```python
from build123d import *

# Parameters (mm, degrees)
BOSS_EXTRUDE1_DEPTH       = 9
BOSS_EXTRUDE1_DEPTH_BACK  = 9
SKETCH1_R                 = 5.25
M4X0_7_TAPPED_HOLE2_D     = 3.3
M4X0_7_TAPPED_HOLE2_DEPTH = 7.1
M4X0_7_TAPPED_HOLE2_TIP   = 0.991420021


with BuildPart() as part:
    # Sketch1 → Boss-Extrude1 (new, two sides: drawn at the far end of the back side and taken through both)
    with BuildSketch(Plane(origin=(0, 0, 0), x_dir=(1, 0, 0), z_dir=(0, 1, 0)).offset(-BOSS_EXTRUDE1_DEPTH_BACK)):
        with BuildLine():
            Line((0, 0), (0, -115))
            Line((0, -115), (2, -115))
            Line((2, -115), (14.5, -95))
            Line((14.5, -95), (30, 2.863148477))
            ThreePointArc((30, 2.863148477), (29.226286483, 10.190585207), (25.056843998, 16.265592284))
            Line((25.056843998, 16.265592284), (25.056843998, 40))
            ThreePointArc((25.056843998, 40), (16.056843998, 49), (7.056843998, 40))
            Line((7.056843998, 40), (7.056843998, 17.036728487))
            Line((7.056843998, 17.036728487), (0, 0))
        make_face()
        with Locations(Location((16.056843998, 40, 0), (0, 0, 270))):
            Circle(SKETCH1_R, mode=Mode.SUBTRACT)
        with Locations(Location((15.152984624, 5, 0), (0, 0, 270))):
            Circle(SKETCH1_R, mode=Mode.SUBTRACT)
    extrude(amount=BOSS_EXTRUDE1_DEPTH + BOSS_EXTRUDE1_DEPTH_BACK)

    # M4x0.7 Tapped Hole2
    with Locations(Plane(origin=(0, 0, 60), x_dir=(0, 0, -1), z_dir=(-1, 0, 0))):
        with Locations((0, 0), (-48, 0)):
            Hole(M4X0_7_TAPPED_HOLE2_D / 2, depth=M4X0_7_TAPPED_HOLE2_DEPTH)
            with Locations((0, 0, -(M4X0_7_TAPPED_HOLE2_DEPTH + M4X0_7_TAPPED_HOLE2_TIP / 2))):  # 118° drill point
                Cone(0, M4X0_7_TAPPED_HOLE2_D / 2, M4X0_7_TAPPED_HOLE2_TIP, mode=Mode.SUBTRACT)


solid = part.part
```
Work out the finished part from the listing and answer in its coordinate system (mm). A direction names the side the tool comes from. Give positions to 0.01 mm unless a question says otherwise; leave off trailing zeros. Order: outer loops, then holes, each group sorted by start corner. A loop starts at its lowest first (then second) coordinate and runs counter-clockwise, first axis right, second up. Notation, with made-up numbers: M 12.5,-32 L 25.5,-32 A14 cw 25.5,-14 Z; hole C -37.75,-1 d8. An arc over 180 degrees is marked long. Return JSON: item names as keys, results as strings.
1) Straight lines are drawn through the part: line 1 along Z through (x, y) = (4, 0.75); line 2 along Y through (x, z) = (3.75, 60); line 3 along Z through (x, y) = (13, -7.5). For each, find the intervals that lie inside material, in ascending order. Write a range as [from, to].
Resolved:
{"line 1": "[-9.66, 58.53], [61.47, 106.53], [109.47, 111.8]", "line 2": "[-9, -1.65], [1.65, 9]", "line 3": "[-48.46, -44.27], [-35.73, -9.79], [-0.21, 97.4]"}
2) Section A-A, the plane y = 6.5 is taken. Write down the section's boundary in (x, z), plus the area to 3 significant figures.
Resolved:
{"outline": "M 0,0 L 7.06,-17.04 L 7.06,-40 A9 ccw 25.06,-40 L 25.06,-16.27 A15 ccw 30,-2.86 L 14.5,95 L 2,115 L 0,115 Z; hole C 15.15,-5 d10.5; hole C 16.06,-40 d10.5", "area": "3,060 mm^2"}
3) Each of these flat-tipped pins is pushed along its axis until it touches: pin 1 (1 mm diameter, centred on x = 10.5, y = 4, fed in from +Z); pin 2 (1.5 mm diameter, centred on y = 1, z = -8, fed in from -X); pin 3 (4 mm diameter, centred on x = 3.5, y = 0.5, fed in from -Z). Where does it stop, or does it pass through?
Resolved:
{"pin 1": "z = 102.2", "pin 2": "x = 3", "pin 3": "z = -13.28"}
4) Section D-D, the plane x = 27.5 is taken. Write down the section's boundary in (y, z), plus the area to 3 significant figures.
Resolved:
{"outline": "M -9,-13.52 L 9,-13.52 L 9,12.92 L -9,12.92 Z", "area": "476 mm^2"}
5) Section B-B, the plane z = -5 is taken. Write down the section's boundary in (x, y).
Resolved:
{"outline": "M 2.07,-9 L 9.9,-9 L 9.9,9 L 2.07,9 Z; M 20.4,-9 L 30.15,-9 L 30.15,9 L 20.4,9 Z"}
6) A tool of negligible diameter and unlimited length cuts with its end or side. For faces 1 (the flat face through (7.057, 0, -29)), 2 (the flat face through (25.057, 0, -28)), 3 (the cylindrical face through (3.6, -0.07, 58.35)), from which of +Z, -Z, +X, -X, +Y, -Y can it reach the whole face along a straight path? Write none if from no direction.
Resolved:
{"face 1": "-Z, -X, +Y, -Y", "face 2": "-Z, +X, +Y, -Y", "face 3": "-X"}
7) Section C-C, the plane z = -31.5 is taken. Write down the section's boundary in (x, y).
Resolved:
{"outline": "M 7.06,-9 L 25.06,-9 L 25.06,9 L 7.06,9 Z"}
8) For a pull along Y with two mould halves and no side action, classify faces 4 (the flat face through (12, -9, 32)), 5 (the flat face through (0, 0, 57)), 6 (the flat face through (12, 9, 32)), 7 (the conical face through (7.9, -0.1, 59.7)) as +Y half, -Y half, draft (parallel to the pull), parting line (faces both ways), or undercut.
Resolved:
{"face 4": "-Y half", "face 5": "draft", "face 6": "+Y half", "face 7": "undercut"}
